Verification items for the finished model (mm, model axes). A direction names the side the tool comes from. Coordinates: 2 decimals unless noted, no trailing zeros. Write each loop counter-clockwise with the first axis right and the second up, starting at its lowest first coordinate (ties: lowest second). Pieces come first, ordered by that corner, then holes. Notation, with made-up numbers: (77, 62) -> (98, 62) arc R20 ccw to (98, 74) -> close; hole circle Ø11 at (36.25, 0.5). An arc over 180 degrees is marked (long way). Answer in a Markdown table with one row per item.
```python
from build123d import *

# Parameters (mm, degrees)
BASE_BLOCK_PROFILE_W         = 61
BASE_BLOCK_PROFILE_H         = 41
BASE_BLOCK_41X61X120_DEPTH   = 120
LENGTHWISE_STEP_CUT_DEPTH    = 120
CASTELLATED_END_BOSSES_DEPTH = 11
TAPERED_NOSE_CUT_DEPTH       = 128.759539761
TAPERED_NOSE_CUT_DEPTH_BACK  = 51
TAPERED_NOSE_PROFILE_W       = 10
TAPERED_NOSE_PROFILE_H       = 86.04422701
TAPERED_NOSE_PROFILE_W_2     = 10.506122453
NOSE_SLOT_CUT_DEPTH          = 51
CROSS_HOLE_DEPTH             = 128.759539761
CROSS_HOLE_DEPTH_BACK        = 128.759539761
CROSS_HOLE_PROFILE_R         = 5.5


with BuildPart() as part:
    # Base Block Profile → Base Block 41x61x120 (new body)
    with BuildSketch(Plane.XY):
        Rectangle(BASE_BLOCK_PROFILE_W, BASE_BLOCK_PROFILE_H)
    extrude(amount=BASE_BLOCK_41X61X120_DEPTH)

    # Step Cut Profile → Lengthwise Step Cut (cut)
    with BuildSketch(Plane(origin=(30.5, 0, 0), x_dir=(0, 0, -1), z_dir=(1, 0, 0))):
        Polygon((-22, -3.5), (0, -3.5), (0, 20.5), (-92, 20.5), (-92, 8.5), (-22, 8.5), align=None)
    extrude(amount=-LENGTHWISE_STEP_CUT_DEPTH, mode=Mode.SUBTRACT)

    # End Boss Profile → Castellated End Bosses (add)
    with BuildSketch(Plane(origin=(0, 20.5, 0), x_dir=(1, 0, 0), z_dir=(0, 1, 0))):
        Polygon((-19, -120), (-30.5, -120), (-30.5, -92), (-11.5, -92), (-11.5, -110), (-19, -110), align=None)
        Polygon((11.5, -92), (30.5, -92), (30.5, -120), (19, -120), (19, -110), (11.5, -110), align=None)
    extrude(amount=CASTELLATED_END_BOSSES_DEPTH)

    # Tapered Nose Profile → Tapered Nose Cut (cut, two sides: drawn at the far end of the back side and taken through both)
    with BuildSketch(Plane(origin=(0, 0, 0), x_dir=(1, 0, 0), z_dir=(0, 1, 0)).offset(-TAPERED_NOSE_CUT_DEPTH_BACK)):
        with Locations((-25.5, -48.977886495)):
            Rectangle(TAPERED_NOSE_PROFILE_W, TAPERED_NOSE_PROFILE_H)
        with Locations((25.246938774, -48.977886495)):
            Rectangle(TAPERED_NOSE_PROFILE_W_2, TAPERED_NOSE_PROFILE_H)
        Polygon((19.993877547, -5.95577299), (3.898702125, -5.95577299), (19.993877547, -38.95577299), align=None)
        Polygon((-20.5, -38.95577299), (-4.404824577, -5.95577299), (-20.5, -5.95577299), align=None)
    extrude(amount=TAPERED_NOSE_CUT_DEPTH + TAPERED_NOSE_CUT_DEPTH_BACK, mode=Mode.SUBTRACT)

    # Nose Slot Profile → Nose Slot Cut (cut)
    with BuildSketch(Plane(origin=(0, -3.5, 0), x_dir=(1, 0, 0), z_dir=(0, 1, 0))):
        Polygon((-30.5, -5.95577299), (3.898702125, -5.95577299), (30.5, -5.95577299), (30.5, 0), (-30.5, 0), align=None)
    extrude(amount=-NOSE_SLOT_CUT_DEPTH, mode=Mode.SUBTRACT)

    # Cross Hole Profile → Cross Hole (cut, two sides: drawn at the far end of the back side and taken through both)
    with BuildSketch(Plane(origin=(0, 0, 0), x_dir=(0, 0, -1), z_dir=(1, 0, 0)).offset(-CROSS_HOLE_DEPTH_BACK)):
        with Locations(Location((-38.95577299, -3.5, 0), (0, 0, 90))):
            Circle(CROSS_HOLE_PROFILE_R)
    extrude(amount=CROSS_HOLE_DEPTH + CROSS_HOLE_DEPTH_BACK, mode=Mode.SUBTRACT)


solid = part.part
```
1. Material ranges on probe 1 along Z at (x, y) = (-2, -3); probe 2 along X at (y, z) = (23, 97); probe 3 along Y at (x, z) = (1.5, 85), recorded low to high. Write a range as from..to.
Findings below:
| item | result |
|---|---|
| probe 1 | z = 22..33.48, 44.43..120 |
| probe 2 | x = -30.5..-11.5, 11.5..30.5 |
| probe 3 | y = -20.5..8.5 |
2. Access from +Z, -Z, +X, -X, +Y, -Y to the whole of each face (thin tool, end or side, straight path). Record for faces 5 (the face through (15, 26, 110)), 6 (the face through (0, -3.5, 16)), 7 (the face through (-11.5, 26, 101)), 8 (the face through (19.994, -6, 66)).
Findings below:
| item | result |
|---|---|
| face 5 | +Z, +Y |
| face 6 | -Z, +X, -X, +Y |
| face 7 | +Z, -Z, +Y |
| face 8 | -Z, +X, +Y, -Y |
3. Go/stop test with flat-tipped pins: pin 1 (13 mm diameter, centred on x = 5.5, y = 0.5, fed in from -Z); pin 2 (14.5 mm diameter, centred on y = 0.5, z = 72, fed in from -X); pin 3 (17.5 mm diameter, centred on x = 1, z = 14, fed in from +Y); pin 4 (1.5 mm diameter, centred on y = -8, z = 45.5, fed in from +X). Record where each tip stops, or that it passes through.
Findings below:
| item | result |
|---|---|
| pin 1 | stops at z = 5.96 |
| pin 2 | stops at x = -20.5 |
| pin 3 | stops at y = 8.5 |
| pin 4 | stops at x = 19.99 |
4. Sectioned sample at D-D, the plane y = -1. Record the cut outline in (x, z).
Findings below:
| item | result |
|---|---|
| outline | (-30.5, 92) -> (-20.5, 92) -> (-20.5, 43.85) -> (19.99, 43.85) -> (19.99, 92) -> (30.5, 92) -> (30.5, 120) -> (-30.5, 120) -> close; (-18.11, 34.06) -> (-12.23, 22) -> (11.72, 22) -> (17.6, 34.06) -> close |
5. Sectioned sample at B-B, the plane z = 100. Record the cut outline in (x, y), and give its area (3 significant figures).
Findings below:
| item | result |
|---|---|
| outline | (-30.5, -20.5) -> (30.5, -20.5) -> (30.5, 31.5) -> (11.5, 31.5) -> (11.5, 20.5) -> (-11.5, 20.5) -> (-11.5, 31.5) -> (-30.5, 31.5) -> close |
| area | 2,920 mm² |
6. Release check for a two-part mould opening along X. For faces 1 (the face through (0, -12, 5.956)), 2 (the face through (-12.565, -9.425, 22.687)), 3 (the face through (-19, 26, 115)), 4 (the face through (19, 26, 115)) record: released by +X, released by -X, zero draft, split by the parting line, or undercut.
Findings below:
| item | result |
|---|---|
| face 1 | zero draft |
| face 2 | released by -X |
| face 3 | undercut |
| face 4 | undercut |
7. Sectioned sample at A-A, the plane y = -11. Record the cut outline in (x, z).
Findings below:
| item | result |
|---|---|
| outline | (-30.5, 92) -> (-20.5, 92) -> (-20.5, 38.96) -> (-4.4, 5.96) -> (3.9, 5.96) -> (19.99, 38.96) -> (19.99, 92) -> (30.5, 92) -> (30.5, 120) -> (-30.5, 120) -> close |
8. Sectioned sample at C-C, the plane x = -9.5. Record the cut outline in (y, z).
Findings below:
| item | result |
|---|---|
| outline | (-20.5, 16.4) -> (-3.5, 16.4) -> (-3.5, 22) -> (8.5, 22) -> (8.5, 92) -> (20.5, 92) -> (20.5, 120) -> (-20.5, 120) -> close; hole circle Ø11 at (-3.5, 38.96) |
